CAD build for the part. Positions are in the model's coordinates, mm. A direction names the side the tool comes from. Coordinates: 2 decimals unless noted, no trailing zeros. Order: outer loops, then holes, each group sorted by start corner. A loop starts at its lowest first (then second) coordinate and runs counter-clockwise, first axis right, second up. Notation, with made-up numbers: M 25.5,-15 L 78.5,-15 A14 cw 78.5,11 Z; hole C 21,58 d8. An arc over 180 degrees is marked long. Write item = value, one per line. Start each with the question number.
```python
from build123d import *

# Parameters (mm, degrees)
CLEVIS_BLOCK_DEPTH         = 22.5
COUNTERBORE_SKETCH_R       = 12
PIN_HOLE_COUNTERBORE_DEPTH = 9
PIN_HOLE_SKETCH_R          = 6
PIN_HOLE_12_DEPTH          = 21
MOUNTING_ARM_DEPTH         = 30
ARM_CLEARANCE_CUT_DEPTH    = 30
EYE_PROFILE_CUT_DEPTH      = 30
EYE_BORE_SKETCH_R          = 7.5
EYE_BORE_DEPTH             = 30
RELIEF_SLOT_CUT_DEPTH      = 148.549271396
RELIEF_SLOT_CUT_DEPTH_BACK = 148.549271396


with BuildPart() as part:
    # Clevis Block Sketch → Clevis Block (new, symmetric)
    with BuildSketch(Plane.XY):
        with BuildLine():
            Line((0, -30), (-60, -30))
            Line((-60, -30), (-60, -9))
            Line((-60, -9), (-28.618176043, -9))
            Line((-28.618176043, -9), (-12, -9))
            ThreePointArc((-12, -9), (15, 0), (-12, 9))
            Line((-12, 9), (-28.618176043, 9))
            Line((-28.618176043, 9), (-60, 9))
            Line((-60, 9), (-60, 30))
            Line((-60, 30), (0, 30))
            ThreePointArc((0, 30), (30, 0), (0, -30))
        make_face()
    extrude(amount=CLEVIS_BLOCK_DEPTH, both=True)

    # Counterbore Sketch → Pin Hole Counterbore (cut)
    with BuildSketch(Plane(origin=(0, 30, 0), x_dir=(1, 0, 0), z_dir=(0, 1, 0))):
        with Locations(Location((-30, 0, 0), (0, 0, 180))):
            Circle(COUNTERBORE_SKETCH_R)
    pin_hole_counterbore = extrude(amount=-PIN_HOLE_COUNTERBORE_DEPTH, mode=Mode.SUBTRACT)

    # Pin Hole Sketch → Pin Hole Ø12 (cut)
    with BuildSketch(Plane(origin=(0, 30, 0), x_dir=(1, 0, 0), z_dir=(0, 1, 0))):
        with Locations(Location((-30, 0, 0), (0, 0, 180))):
            Circle(PIN_HOLE_SKETCH_R)
    pin_hole_12 = extrude(amount=-PIN_HOLE_12_DEPTH, mode=Mode.SUBTRACT)

    # Counterbore Mirror: Pin Hole Counterbore across plane
    add(pin_hole_counterbore.mirror(Plane.ZX), mode=Mode.SUBTRACT)

    # Pin Hole Mirror: Pin Hole Ø12 across plane
    add(pin_hole_12.mirror(Plane.ZX), mode=Mode.SUBTRACT)

    # Mounting Arm Sketch → Mounting Arm (add, symmetric)
    with BuildSketch(Plane(origin=(0, 0, 0), x_dir=(1, 0, 0), z_dir=(0, 1, 0))):
        Polygon((0, -4.5), (90, -4.5), (137.279960262, 42.779960262), (132.779960262, 47.279960262), (90, 4.5), (0, 4.5), align=None)
    extrude(amount=MOUNTING_ARM_DEPTH, both=True)

    # Arm Clearance Cut Sketch → Arm Clearance Cut (cut, symmetric)
    with BuildSketch(Plane(origin=(0, 0, -4.5), x_dir=(-1, 0, 0), z_dir=(0, 0, -1))):
        with BuildLine():
            Line((-51, 21), (-51, 30))
            Line((-51, 30), (-60, 30))
            Line((-60, 30), (-69, 30))
            Line((-69, 30), (-69, 0))
            ThreePointArc((-69, 0), (-60, -9), (-51, 0))
            Line((-51, 0), (-51, 21))
        make_face()
    extrude(amount=ARM_CLEARANCE_CUT_DEPTH, both=True, mode=Mode.SUBTRACT)

    # Eye Profile Cut Sketch → Eye Profile Cut (cut, symmetric)
    with BuildSketch(Plane(origin=(42.75, 0, 42.75), x_dir=(-0.7071067811865513, 0, 0.7071067811865437), z_dir=(-0.7071067811865437, 0, -0.7071067811865513))):
        with BuildLine():
            Line((-127.321590822, 30), (-127.321590822, 0))
            ThreePointArc((-127.321590822, 0), (-124.412282123, 8.87779161), (-116.812899639, 14.311818372))
            Line((-116.812899639, 14.311818372), (-66.821590822, 30))
            Line((-66.821590822, 30), (-127.321590822, 30))
        make_face()
        with BuildLine():
            ThreePointArc((-116.812899639, -14.311818372), (-124.412282123, -8.87779161), (-127.321590822, 0))
            Line((-127.321590822, 0), (-127.321590822, -30))
            Line((-127.321590822, -30), (-66.821590822, -30))
            Line((-66.821590822, -30), (-116.812899639, -14.311818372))
        make_face()
    extrude(amount=EYE_PROFILE_CUT_DEPTH, both=True, mode=Mode.SUBTRACT)

    # Eye Bore Sketch → Eye Bore (cut, symmetric)
    with BuildSketch(Plane(origin=(42.75, 0, 42.75), x_dir=(-0.7071067811865513, 0, 0.7071067811865437), z_dir=(-0.7071067811865437, 0, -0.7071067811865513))):
        with Locations((-112.321590822, 0)):
            Circle(EYE_BORE_SKETCH_R)
    extrude(amount=EYE_BORE_DEPTH, both=True, mode=Mode.SUBTRACT)

    # Relief Slot Sketch → Relief Slot Cut (cut, two sides: drawn at the far end of the back side and taken through both)
    with BuildSketch(Plane(origin=(0, 0, -22.5), x_dir=(-1, 0, 0), z_dir=(0, 0, -1)).offset(-RELIEF_SLOT_CUT_DEPTH_BACK)):
        with BuildLine():
            Line((0, 15), (0, -15))
            ThreePointArc((0, -15), (-15, 0), (0, 15))
        make_face()
    extrude(amount=RELIEF_SLOT_CUT_DEPTH + RELIEF_SLOT_CUT_DEPTH_BACK, mode=Mode.SUBTRACT)


solid = part.part
```
1. Probe L1, parallel to Z at x = -30, y = -17; L2, parallel to Y at x = -30, z = 12.5; L3, parallel to Z at x = -50.5, y = 20. List the from-to ranges inside material, lowest first.
2. Mould opens along Y. For faces 4 (the flat face through (-18, -30, -5)), 5 (the cylindrical face through (-24, 15, 0)), 6 (the cylindrical face through (129.69, 0.33, -39.753)), 7 (the cylindrical face through (29.993, 0.66, 13.626)) say: released by +Y, released by -Y, zero draft, split by the parting line, or undercut.
3. Flat gauge pins, fed straight in: pin 1 (1.5 mm diameter, centred on x = 19, y = 0.5, fed in from -Z); pin 2 (4 mm diameter, centred on x = 52.5, y = -13.5, fed in from +Z); pin 3 (10 mm diameter, centred on y = -20, z = 8, fed in from +X). Where does each tip first touch, or does it go through?
4. 3-axis set-ups, long thin cutter, end or side, ignore diameter. For faces 1 (the flat face through (69, 15, 0)), 2 (the flat face through (-36.3, -9, 0.3)), 3 (the cylindrical face through (-41.085, 25.563, -4.596)): which of +Z, -Z, +X, -X, +Y, -Y reach the whole face in a straight line?
5. Slice it at B-B (y = -12). Write the cut outline in (x, z).
6. Slice it at D-D (y = 18). Write the cut outline in (x, z), plus the area to 3 significant figures.
7. Slice it at C-C (z = 14). Write the cut outline in (x, y).
8. Slice it at A-A (x = -30). Write the cut outline in (y, z).
Calculated:
q1.L1 = -22.5 to -6, 6 to 22.5
q1.L2 = -30 to -9, 9 to 30
q1.L3 = -22.5 to 22.5
q2.face_4 = released by -Y
q2.face_5 = zero draft
q2.face_6 = undercut
q2.face_7 = split by the parting line
q3.pin_1 = -22.5
q3.pin_2 = 4.5
q3.pin_3 = 91.5
q4.face_1 = +Z, -Z, +Y
q4.face_2 = +Z, -Z, -X
q4.face_3 = +Y
q5.outline = M -60,-22.5 L -9,-22.5 L -9,22.5 L -60,22.5 Z; M 9,-22.5 L 27.5,-22.5 L 27.5,-4.5 L 90,-4.5 L 128.54,-43.04 L 133.04,-38.54 L 90,4.5 L 27.5,4.5 L 27.5,22.5 L 9,22.5 Z; hole C -30,0 d12
q6.outline = M -60,-22.5 L 24,-22.5 L 24,-4.5 L 51,-4.5 L 51,4.5 L 24,4.5 L 24,22.5 L -60,22.5 Z; M 69,-4.5 L 90,-4.5 L 117.04,-31.54 L 121.54,-27.04 L 90,4.5 L 69,4.5 Z; hole C -30,0 d12
q6.area = 4,360 mm²
q7.outline = M -60,-30 L 0,-30 A30 ccw 0,30 L -60,30 L -60,9 L -12,9 A15 cw long -12,-9 L -60,-9 Z
q8.outline = M -30,-22.5 L -9,-22.5 L -9,-6 L -21,-6 L -21,-12 L -30,-12 Z; M -30,12 L -21,12 L -21,6 L -9,6 L -9,22.5 L -30,22.5 Z; M 9,-22.5 L 30,-22.5 L 30,-12 L 21,-12 L 21,-6 L 9,-6 Z; M 9,6 L 21,6 L 21,12 L 30,12 L 30,22.5 L 9,22.5 Z
